Read the model definition and answer for the solid it produces. Units are mm, in the model's axes. Face numbers are marked on the shaded views. A direction names the side the tool comes from. Round coordinates to 2 decimals unless told otherwise and drop trailing zeros. Order: outer loops, then holes, each group sorted by start corner. A loop starts at its lowest first (then second) coordinate and runs counter-clockwise, first axis right, second up. Notation, with made-up numbers: (-39.75, 31.25) - (-4.75, 31.25) arc R28 cw to (-4.75, 54.25) - close; hole circle Ø7 at (85.25, 30.5). An arc over 180 degrees is marked (long way). One line per question, with ' | ' between items. Start each with the question number.
1) The mould has two halves that part along X. Classify the marked faces 1, 2 and 3: pulls with the +X half, pulls with the -X half, needs draft (parallel to the pull), parting line crosses it, or undercut.
2) Flat-ended cylindrical pins translate along their axes: pin 1 (10 mm diameter, centred on x = 20, z = 0, fed in from -Y); pin 2 (9 mm diameter, centred on x = -19, z = -3.5, fed in from +Y). Find the tip coordinate at first contact, or state that the pin passes through.
3) For the marked faces 4 and 5, determine the directions among +Z, -Z, +X, -X, +Y, -Y from which every point of the face is accessible in a straight line to the end or side of a thin tool.
4) Straight lines are drawn through the part: line 1 (X direction, y = 41, z = 0); line 2 (X direction, y = 26, z = 0); line 3 (Z direction, x = -20, y = 16). For each, find the intervals that lie inside material, in ascending order. Write a range as from..to.
5) The part is cut by section C-C, the plane y = 46. Give the vertices of the cut face in (x, z).
6) The part is cut by section A-A, the plane x = -20. Give the vertices of the cut face in (y, z).
7) The part is cut by section B-B, the plane z = 0. Give the vertices of the cut face in (x, y).
8) The part is cut by section D-D, the plane z = -7. Give the vertices of the cut face in (x, y).
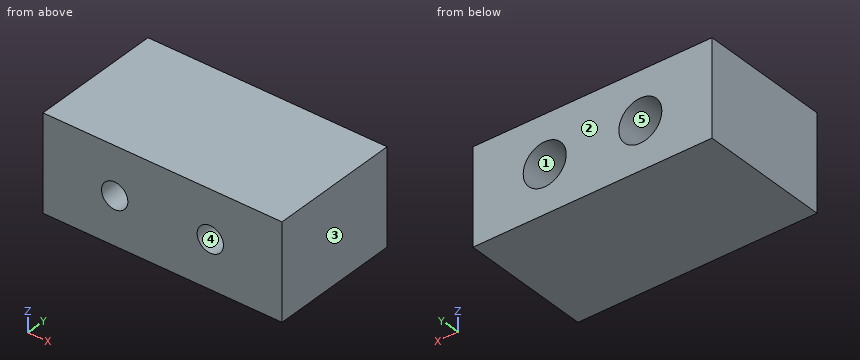
from build123d import *

# Parameters (mm, degrees)
SKETCH1_W           = 100
SKETCH1_H           = 40
SKETCH1_R           = 5.5
BOSS_EXTRUDE1_DEPTH = 55
SKETCH2_R           = 9
CUT_EXTRUDE1_DEPTH  = 20


with BuildPart() as part:
    # Sketch1 → Boss-Extrude1 (new body)
    with BuildSketch(Plane(origin=(0, 0, 0), x_dir=(1, 0, 0), z_dir=(0, 1, 0))):
        Rectangle(SKETCH1_W, SKETCH1_H)
        with Locations(Location((-20, 0, 0), (0, 0, 270))):
            Circle(SKETCH1_R, mode=Mode.SUBTRACT)
        with Locations(Location((20, 0, 0), (0, 0, 270))):
            Circle(SKETCH1_R, mode=Mode.SUBTRACT)
    extrude(amount=BOSS_EXTRUDE1_DEPTH)

    # Sketch2 → Cut-Extrude1 (cut)
    with BuildSketch(Plane(origin=(0, 55, 0), x_dir=(1, 0, 0), z_dir=(0, 1, 0))):
        with Locations(Location((20, 0, 0), (0, 0, 270))):
            Circle(SKETCH2_R)
        with Locations(Location((-20, 0, 0), (0, 0, 270))):
            Circle(SKETCH2_R)
    extrude(amount=-CUT_EXTRUDE1_DEPTH, mode=Mode.SUBTRACT)


solid = part.part
Values:
1) face 1: undercut | face 2: needs draft | face 3: pulls with the +X half
2) pin 1: passes through | pin 2: stops at y = 35
3) face 4: +Y, -Y | face 5: +Y
4) line 1: x = -50..-29, -11..11, 29..50 | line 2: x = -50..-25.5, -14.5..14.5, 25.5..50 | line 3: z = -20..-5.5, 5.5..20
5) outline: (-50, -20) - (50, -20) - (50, 20) - (-50, 20) - close; hole circle Ø18 at (-20, 0); hole circle Ø18 at (20, 0)
6) outline: (0, -20) - (55, -20) - (55, -9) - (35, -9) - (35, -5.5) - (0, -5.5) - close; (0, 5.5) - (35, 5.5) - (35, 9) - (55, 9) - (55, 20) - (0, 20) - close
7) outline: (-50, 0) - (-25.5, 0) - (-25.5, 35) - (-29, 35) - (-29, 55) - (-50, 55) - close; (-14.5, 0) - (14.5, 0) - (14.5, 35) - (11, 35) - (11, 55) - (-11, 55) - (-11, 35) - (-14.5, 35) - close; (25.5, 0) - (50, 0) - (50, 55) - (29, 55) - (29, 35) - (25.5, 35) - close
8) outline: (-50, 0) - (50, 0) - (50, 55) - (25.66, 55) - (25.66, 35) - (14.34, 35) - (14.34, 55) - (-14.34, 55) - (-14.34, 35) - (-25.66, 35) - (-25.66, 55) - (-50, 55) - close
